from build123d import *

# Parameters (mm, degrees)
SKETCH1_R           = 15.75
SKETCH1_R_2         = 9.5
BOSS_EXTRUDE1_DEPTH = 4
SKETCH3_R           = 10.639095477
SKETCH3_R_2         = 8.5
BOSS_EXTRUDE2_DEPTH = 2
M3_TAPPED_HOLE1_D   = 2.5
CHAMFER1_SIZE       = 0.2
SKETCH6_R           = 20.677002962
SKETCH6_R_2         = 13.25
CUT_EXTRUDE1_DEPTH  = 0.45
CHAMFER2_SIZE       = 0.5


with BuildPart() as part:
    # Sketch1 → Boss-Extrude1 (new, symmetric)
    with BuildSketch(Plane.XY):
        Circle(SKETCH1_R)
        Circle(SKETCH1_R_2, mode=Mode.SUBTRACT)
    extrude(amount=BOSS_EXTRUDE1_DEPTH, both=True)

    # Sketch3 → Boss-Extrude2 (add)
    with BuildSketch(Plane(origin=(0, 0, -4), x_dir=(-1, 0, 0), z_dir=(0, 0, -1))):
        Circle(SKETCH3_R)
        Circle(SKETCH3_R_2, mode=Mode.SUBTRACT)
    extrude(amount=-BOSS_EXTRUDE2_DEPTH)

    # M3 Tapped Hole1 (through all)
    with Locations(Plane.XY.offset(4)):
        with Locations((0, -11.5)):
            m3_tapped_hole1 = Hole(M3_TAPPED_HOLE1_D / 2)

    # Mirror1: M3 Tapped Hole1 across plane
    add(m3_tapped_hole1.mirror(Plane.ZX), mode=Mode.SUBTRACT)

    # Chamfer1
    chamfer1_edges = [part.edges().sort_by_distance(p)[0] for p in [
        (-9.5, 0, 4),
    ]]
    chamfer(chamfer1_edges, length=CHAMFER1_SIZE)

    # Sketch6 → Cut-Extrude1 (cut)
    with BuildSketch(Plane.XY.offset(4)):
        Circle(SKETCH6_R)
        Circle(SKETCH6_R_2, mode=Mode.SUBTRACT)
    extrude(amount=-CUT_EXTRUDE1_DEPTH, mode=Mode.SUBTRACT)

    # Chamfer2
    chamfer2_edges = [part.edges().sort_by_distance(p)[0] for p in [
        (-15.75, 0, -4),
    ]]
    chamfer(chamfer2_edges, length=CHAMFER2_SIZE)


solid = part.part
Design review of the part built by this model. Coordinates are the model's own, in mm. A direction names the side the tool comes from. Give positions to 0.01 mm unless a question says otherwise; leave off trailing zeros. Loops run counter-clockwise (first coordinate to the right, second up) from the corner with the lowest first, then second, coordinate; pieces in that order, holes last. Notation, with made-up numbers: M 61,7 L 120,7 A22 cw 120,30 Z; hole C 54.5,-18.75 d3. An arc over 180 degrees is marked long. Answer as a JSON object with one key per item and string values.
Item 1: Wall thickness on line 1 along Y through (x, z) = (0, -3.1); line 2 along Y through (x, z) = (0, -0.45); line 3 along Y through (x, z) = (-8.5, 0.5): over which ranges is each line inside the solid? List them lowest first.
Output values:
{"line 1": "y = -15.75 to -12.75, -10.25 to -8.5, 8.5 to 10.25, 12.75 to 15.75", "line 2": "y = -15.75 to -12.75, -10.25 to -9.5, 9.5 to 10.25, 12.75 to 15.75", "line 3": "y = -13.26 to -4.24, 4.24 to 13.26"}
Item 2: We need section A-A (x = 0). State the section outline as (y, z) points, and give its area (3 significant figures).
Output values:
{"outline": "M -15.75,-3.5 L -15.25,-4 L -12.75,-4 L -12.75,4 L -13.25,4 L -13.25,3.55 L -15.75,3.55 Z; M -10.25,-4 L -8.5,-4 L -8.5,-2 L -9.5,-2 L -9.5,3.8 L -9.7,4 L -10.25,4 Z; M 8.5,-4 L 10.25,-4 L 10.25,4 L 9.7,4 L 9.5,3.8 L 9.5,-2 L 8.5,-2 Z; M 12.75,-4 L 15.25,-4 L 15.75,-3.5 L 15.75,3.55 L 13.25,3.55 L 13.25,4 L 12.75,4 Z", "area": "61.5 mm2"}
Item 3: Machinability: for faces 5 (the face through (2.2, -8.4, -2)), 6 (the face through (-7, -7, 4)), which of the approach directions +Z, -Z, +X, -X, +Y, -Y give a long, thin tool a straight path to every point of the face, cutting with its end or side? Answer none if there is none.
Output values:
{"face 5": "+Z", "face 6": "+Z, +X, -X, +Y, -Y"}
Item 4: We need section B-B (y = 0). State the section outline as (x, z) points, and give its area (3 significant figures).
Output values:
{"outline": "M -15.75,-3.5 L -15.25,-4 L -8.5,-4 L -8.5,-2 L -9.5,-2 L -9.5,3.8 L -9.7,4 L -13.25,4 L -13.25,3.55 L -15.75,3.55 Z; M 8.5,-4 L 15.25,-4 L 15.75,-3.5 L 15.75,3.55 L 13.25,3.55 L 13.25,4 L 9.7,4 L 9.5,3.8 L 9.5,-2 L 8.5,-2 Z", "area": "101 mm2"}
Item 5: We need section C-C (z = -3). State the section outline as (x, y) points, and give its area (3 significant figures).
Output values:
{"outline": "C 0,0 d31.5; hole C 0,0 d17; hole C 0,-11.5 d2.5; hole C 0,11.5 d2.5", "area": "543 mm2"}
Item 6: Mouldability with a two-part tool opening along Y and no side actions: class faces 1 (the face through (0.16, -10.26, -0.06)), 2 (the face through (-0.672, 10.446, -0.056)), 3 (the face through (7.123, 11.172, 3.778)), 4 (the face through (7, -7, -4)) as pulls with the +Y half, pulls with the -Y half, needs draft (parallel to the pull), parting line crosses it, or undercut.
Output values:
{"face 1": "undercut", "face 2": "undercut", "face 3": "parting line crosses it", "face 4": "needs draft"}
Item 7: We need section D-D (z = 3). State the section outline as (x, y) points.
Output values:
{"outline": "C 0,0 d31.5; hole C 0,0 d19; hole C 0,-11.5 d2.5; hole C 0,11.5 d2.5"}
Item 8: For P1, Ø3, axis at y = -2.5, z = 0.5, coming from the +X side, flat-tipped, find the tip position at first contact; note if it passes through.
Output values:
{"P1": "stops at x = 15.72"}
